Check sheet for the modelled part. Datum: model origin and axes. Units: mm. Give positions to 0.01 mm unless a question says otherwise; leave off trailing zeros. Order: outer loops, then holes, each group sorted by start corner. A loop starts at its lowest first (then second) coordinate and runs counter-clockwise, first axis right, second up.
Item 1: Sectioned sample at C-C on y = 24.5. Record the boundary of the cut face in (x, z).
Item 2: Material ranges on line 1 along X through (y, z) = (11, 2.5); line 2 along X through (y, z) = (23, 4.75); line 3 along Y through (x, z) = (7, 5.5), recorded low to high.
Item 3: Sectioned sample at A-A on z = 7. Record the boundary of the cut face in (x, y).
Item 4: Gauge pin test, flat ends, axial feed: P1, Ø6, axis at x = 25.5, z = 2.5, coming from the +Y side; P2, Ø2, axis at y = 22.5, z = 6.5, coming from the +X side; P3, Ø1.5, axis at x = 17, y = 4.5, coming from the -Z side; P4, Ø4, axis at y = 17.5, z = 1.5, coming from the +X side. Record the tip position at first contact, or that the pin passes through.
Item 5: Sectioned sample at B-B on x = 27.25. Record the boundary of the cut face in (y, z), and give its area (3 significant figures).
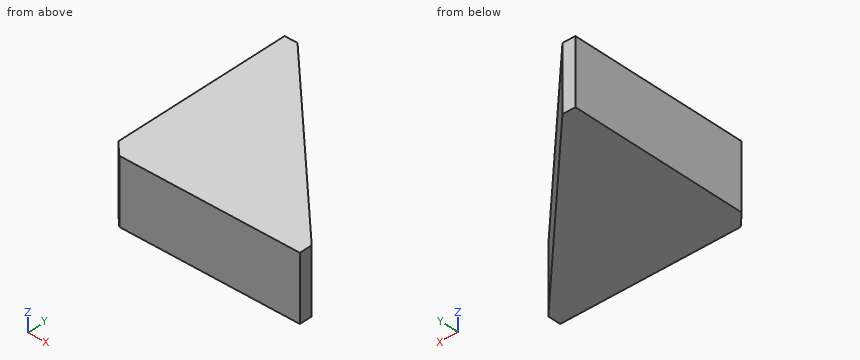
from build123d import *

# Parameters (mm, degrees)
EXTRUDE_1_DEPTH = 10
CHAMFER_1_SIZE  = 2


with BuildPart() as part:
    # 草图1 → 凸台-拉伸1 (new body)
    with BuildSketch(Plane.XY):
        Polygon((0, 30), (0, 0), (30, 0), (30, 2), (2, 30), align=None)
    extrude(amount=EXTRUDE_1_DEPTH)

    # 倒角1
    chamfer_1_edges = [part.edges().sort_by_distance(p)[0] for p in [
        (0, 0, 5),
    ]]
    chamfer(chamfer_1_edges, length=CHAMFER_1_SIZE)


solid = part.part
Report:
1. outline: (0, 0) - (7.5, 0) - (7.5, 10) - (0, 10) - close
2. line 1: x = 0 to 21
2. line 2: x = 0 to 9
2. line 3: y = 0 to 25
3. outline: (0, 2) - (2, 0) - (30, 0) - (30, 2) - (2, 30) - (0, 30) - close
4. P1: stops at y = 9.5
4. P2: stops at x = 10.5
4. P3: stops at z = 0
4. P4: stops at x = 16.5
5. outline: (0, 0) - (4.75, 0) - (4.75, 10) - (0, 10) - close
5. area: 47.5 mm2
